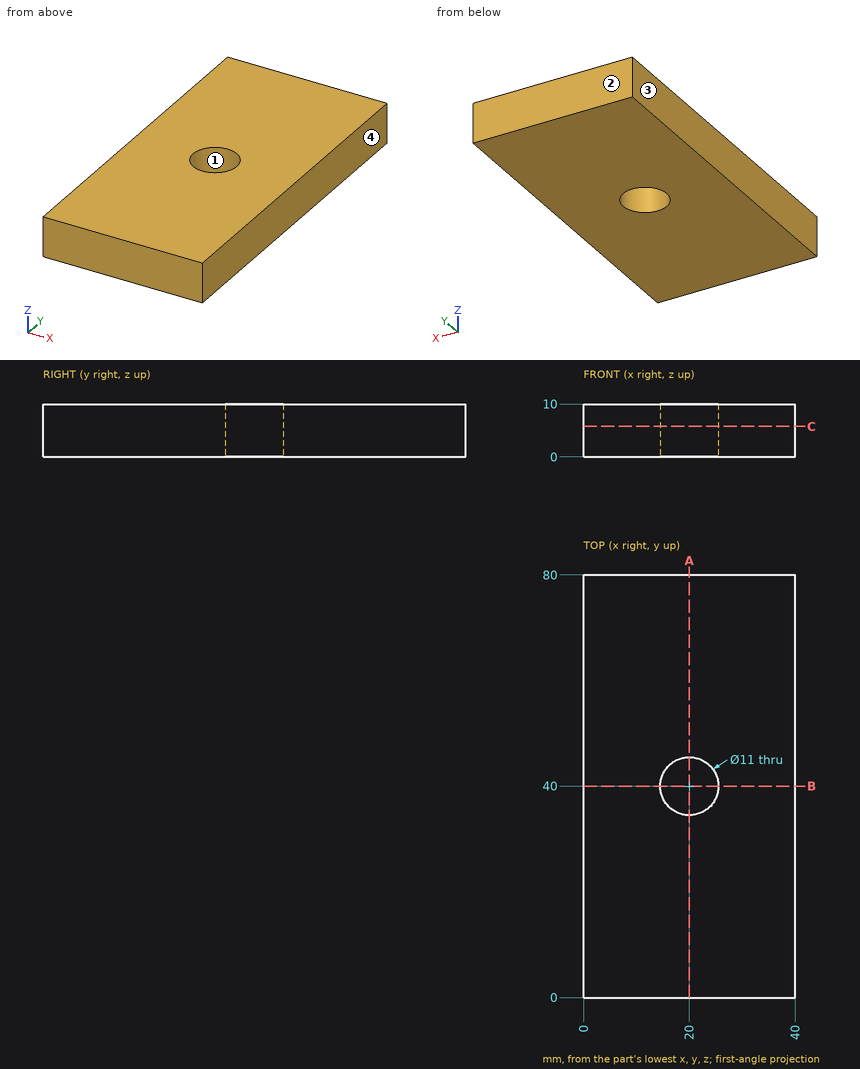
Geometry: see drawing. Coordinates: mm, zero at the bounding-box minimum. Round coordinates to 2 decimals unless told otherwise and drop trailing zeros. Loops run counter-clockwise (first coordinate to the right, second up) from the corner with the lowest first, then second, coordinate; pieces in that order, holes last. Notation, with made-up numbers: (38.25, -2) -> (93.25, -2) arc R11 cw to (93.25, 14) -> close; hole circle Ø10 at (8.25, 23.25). An arc over 180 degrees is marked (long way). Write each question's results on one line, items separated by ' | '.
Item 1: Cut plane C-C on z = 5.75. Return the cut outline in (x, y).
Answers below:
outline: (0, 0) -> (40, 0) -> (40, 80) -> (0, 80) -> close; hole circle Ø11 at (20, 40)
Item 2: Line query: probe 1 along Y at (x, z) = (20, 6.25); probe 2 along X at (y, z) = (44, 9.25); probe 3 along X at (y, z) = (39, 2.5). Output: solid intervals per line, ascending. Write a range as [from, to].
Answers below:
probe 1: y = [0, 34.5], [45.5, 80] | probe 2: x = [0, 16.23], [23.77, 40] | probe 3: x = [0, 14.59], [25.41, 40]
Item 3: Cut plane A-A on x = 20. Return the cut outline in (y, z), and give its area (3 significant figures).
Answers below:
outline: (0, 0) -> (34.5, 0) -> (34.5, 10) -> (0, 10) -> close; (45.5, 0) -> (80, 0) -> (80, 10) -> (45.5, 10) -> close | area: 690 mm²
Item 4: Pull-direction query (X, two-part tool) for the marked faces 1, 2, 3 and 4; classes: pulls with the +X half, pulls with the -X half, needs draft (parallel to the pull), parting line crosses it, or undercut.
Answers below:
face 1: undercut | face 2: needs draft | face 3: pulls with the -X half | face 4: pulls with the +X half
Item 5: Cut plane B-B on y = 40. Return the cut outline in (x, z).
Answers below:
outline: (0, 0) -> (14.5, 0) -> (14.5, 10) -> (0, 10) -> close; (25.5, 0) -> (40, 0) -> (40, 10) -> (25.5, 10) -> close
Item 6: Pin query (flat end, axial travel): pin 1 Ø14.5 at (x, y) = (20, 40) entering from -Z. Return the tip coordinate at first contact, or that it passes through.
Answers below:
pin 1: stops at z = 0
